The listing builds one solid part. Answer for the finished solid, in the listing's coordinates (mm). A direction names the side the tool comes from. Round coordinates to 2 decimals unless told otherwise and drop trailing zeros. Order: outer loops, then holes, each group sorted by start corner. A loop starts at its lowest first (then second) coordinate and runs counter-clockwise, first axis right, second up. Notation, with made-up numbers: (29.5, 32.5) -> (78.5, 32.5) arc R16 cw to (78.5, 46.5) -> close; hole circle Ø1 at (-25, 32). An arc over 180 degrees is marked (long way). Answer in a Markdown table with one row per item. Add a question column.
```python
from build123d import *

# Parameters (mm, degrees)
SKETCH1_R           = 62.5
SKETCH1_R_2         = 57.5
BOSS_EXTRUDE1_DEPTH = 13
SKETCH2_R           = 80
SKETCH2_R_2         = 52.5
BOSS_EXTRUDE2_DEPTH = 12
CUT_EXTRUDE1_START  = -7
SKETCH3_R           = 57.5
CUT_EXTRUDE1_DEPTH  = 7
CIRPATTERN1_COUNT   = 8
CHAMFER1_SIZE       = 1


with BuildPart() as part:
    # Sketch1 → Boss-Extrude1 (new body)
    with BuildSketch(Plane.XY):
        Circle(SKETCH1_R)
        Circle(SKETCH1_R_2, mode=Mode.SUBTRACT)
    extrude(amount=BOSS_EXTRUDE1_DEPTH)

    # Sketch2 → Boss-Extrude2 (add)
    with BuildSketch(Plane(origin=(0, 0, 0), x_dir=(-1, 0, 0), z_dir=(0, 0, -1))):
        Circle(SKETCH2_R)
        Circle(SKETCH2_R_2, mode=Mode.SUBTRACT)
    extrude(amount=BOSS_EXTRUDE2_DEPTH)

    # Sketch3 → Cut-Extrude1 (cut)
    with BuildSketch(Plane.XY.offset(CUT_EXTRUDE1_START)):
        Circle(SKETCH3_R)
    extrude(amount=CUT_EXTRUDE1_DEPTH, mode=Mode.SUBTRACT)

    # Sketch5 → Hole size (%based on) socket head cap screw type1 (revolve, cut)
    with BuildSketch(Plane(origin=(-70, 0, -12), x_dir=(0, 1, 0), z_dir=(1, 0, 0))):
        Polygon((0, 0), (0, 26.482840043), (3.3, 24.5), (3.3, 6.8), (5.5, 6.8), (5.5, 0), align=None)
    hole_size_based_on_socket_head_cap_scr = revolve(axis=Axis((-70, 0, -18.35), (0, 0, 1)), mode=Mode.SUBTRACT)

    # CirPattern1: Hole size (%based on) socket head cap screw type1 ×8 about axis
    cirpattern1_axis = Axis((0, 0, 0), (0, 0, 1))
    for i in range(1, CIRPATTERN1_COUNT):
        add(hole_size_based_on_socket_head_cap_scr.rotate(cirpattern1_axis, i * 360 / CIRPATTERN1_COUNT), mode=Mode.SUBTRACT)

    # Chamfer1
    chamfer1_edges = [part.edges().sort_by_distance(p)[0] for p in [
        (80, 0, -12),
        (80, 0, 0),
        (52.5, 0, -12),
        (52.5, 0, -7),
        (-62.5, 0, 13),
        (-57.5, 0, 13),
    ]]
    chamfer(chamfer1_edges, length=CHAMFER1_SIZE)


solid = part.part
```
1. The mould has two halves that part along X. Classify faces 4 (the flat face through (-35, -52, 0)), 5 (the cylindrical face through (48.5, 46.35, -2.64)), 6 (the cylindrical face through (46.35, -48.5, -2.64)): released by +X, released by -X, zero draft, split by the parting line, or undercut.
2. For faces 1 (the flat face through (-66, 0, -5.2)), 2 (the cylindrical face through (-48.5, -46.35, -2.64)), 3 (the flat face through (17, -51, -7)), determine the directions among +Z, -Z, +X, -X, +Y, -Y from which every point of the face is accessible in a straight line to the end or side of a thin tool.
3. Each of these flat-tipped pins is pushed along its axis until it touches: pin 1 (3.5 mm diameter, centred on x = 51, y = -51, fed in from -Z); pin 2 (10 mm diameter, centred on y = 21.5, z = -8, fed in from -X); pin 3 (12 mm diameter, centred on x = 63.5, z = -8.5, fed in from -Y); pin 4 (6.5 mm diameter, centred on x = 0, y = -70, fed in from +Z). Where does it stop, or does it pass through?
4. The part is cut by section A-A (y = 0). Give the number of separate pieces and of enclosed holes in the cut face, then the cut area to 3 significant figures.
5. The part is cut by section B-B (z = 7.5). Give the vertices of the cut face in (x, y), then the cut area to 3 significant figures.
6. Straight lines are drawn through the part: line 1 along X through (y, z) = (49, -2.5); line 2 along Y through (x, z) = (0.5, 6); line 3 along X through (y, z) = (-2.5, -9.5). For each, find the intervals that lie inside material, in ascending order.
Report:
| question | item | result |
|---|---|---|
| 1 | face 4 | zero draft |
| 1 | face 5 | undercut |
| 1 | face 6 | undercut |
| 2 | face 1 | -Z |
| 2 | face 2 | +Z, -Z |
| 2 | face 3 | +Z |
| 3 | pin 1 | stops at z = -5.2 |
| 3 | pin 2 | stops at x = -78.28 |
| 3 | pin 3 | stops at y = -55.62 |
| 3 | pin 4 | passes through |
| 4 | separate pieces | 4 |
| 4 | enclosed holes | 0 |
| 4 | area | 496 mm^2 |
| 5 | outline | circle Ø125 at (0, 0); hole circle Ø115 at (0, 0) |
| 5 | area | 1,880 mm^2 |
| 6 | line 1 | x = -63.24 to -52.76, -46.24 to -30.09, 30.09 to 46.24, 52.76 to 63.24 |
| 6 | line 2 | y = -62.5 to -57.5, 57.5 to 62.5 |
| 6 | line 3 | x = -79.96 to -74.9, -65.1 to -52.44, 52.44 to 65.1, 74.9 to 79.96 |
